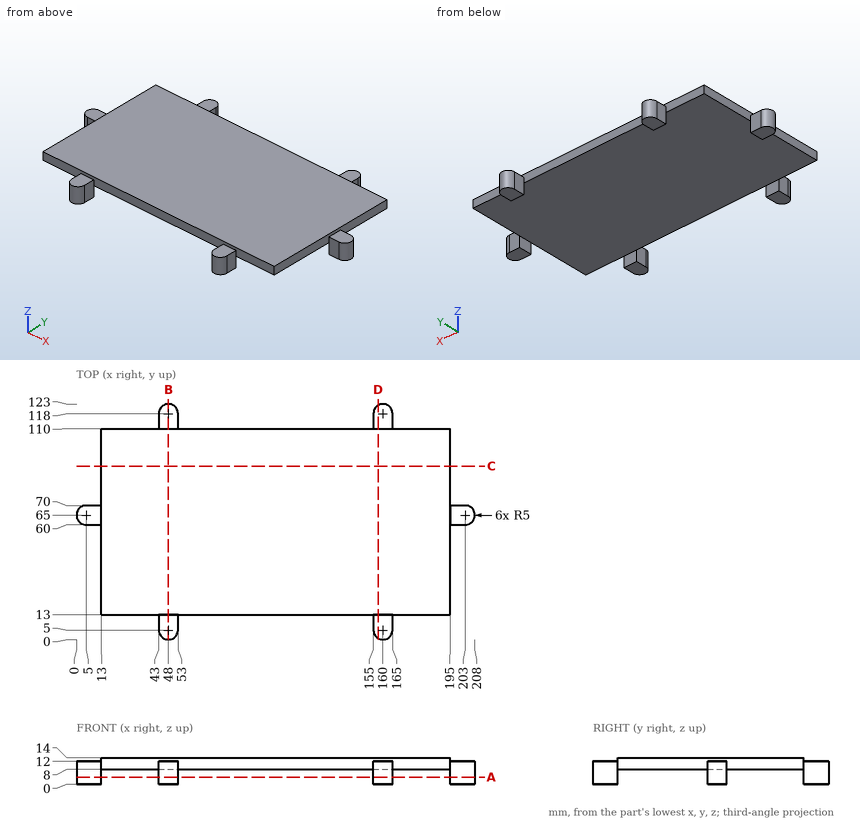
Source: three-view drawing plus pictorial views. Frame: mm from the lowest corner of the part. Round coordinates to 2 decimals unless told otherwise and drop trailing zeros. Loops run counter-clockwise (first coordinate to the right, second up) from the corner with the lowest first, then second, coordinate; pieces in that order, holes last.
Q1. Section B-B on x = 48. Return loops of the section in (y, z), plus the area to 3 significant figures.
Q2. Pin query (flat end, axial travel): P1, Ø4, axis at y = 9, z = 3.5, coming from the -X side; P2, Ø6.5, axis at x = 10.5, z = 8, coming from the +Y side; P3, Ø2.5, axis at x = 201, z = 6, coming from the -Y side. Return the tip coordinate at first contact, or that it passes through.
Q3. Material intervals for L1, parallel to X at y = 12, z = 10.75; L2, parallel to Y at x = 109.5, z = 11; L3, parallel to X at y = 54, z = 13, sorted ascending.
Q4. Section D-D on x = 157.5. Return loops of the section in (y, z).
Q5. Section A-A on z = 3.75. Return loops of the section in (x, y), plus the area to 3 significant figures.
Q6. Section C-C on y = 90.5. Return loops of the section in (x, z), plus the area to 3 significant figures.
Evaluation:
1. outline: (0, 0) - (13, 0) - (13, 8) - (110, 8) - (110, 0) - (123, 0) - (123, 12) - (110, 12) - (110, 14) - (13, 14) - (13, 12) - (0, 12) - close
1. area: 894 mm2
2. P1: stops at x = 43
2. P2: stops at y = 110
2. P3: stops at y = 60
3. L1: x = 43 to 53, 155 to 165
3. L2: y = 13 to 110
3. L3: x = 13 to 195
4. outline: (0.67, 0) - (13, 0) - (13, 8) - (110, 8) - (110, 0) - (122.33, 0) - (122.33, 12) - (110, 12) - (110, 14) - (13, 14) - (13, 12) - (0.67, 12) - close
5. outline: (5, 60) - (13, 60) - (13, 70) - (5, 70) arc R5 ccw to start; (43, 5) arc R5 ccw to (53, 5) - (53, 13) - (43, 13) - close; (43, 110) - (53, 110) - (53, 118) arc R5 ccw to (43, 118) - close; (155, 5) arc R5 ccw to (165, 5) - (165, 13) - (155, 13) - close; (155, 110) - (165, 110) - (165, 118) arc R5 ccw to (155, 118) - close; (195, 60) - (203, 60) arc R5 ccw to (203, 70) - (195, 70) - close
5. area: 716 mm2
6. outline: (13, 8) - (195, 8) - (195, 14) - (13, 14) - close
6. area: 1,090 mm2
